from build123d import *
from build123d.topology import SkipClean

# Parameters (mm, degrees)
BASE_PLATE_DEPTH      = 15
SIDE_BLOCK_A_SKETCH_W = 40
SIDE_BLOCK_A_SKETCH_H = 15
SIDE_BLOCK_A_DEPTH    = 13.5
SIDE_BLOCK_B_SKETCH_W = 40
SIDE_BLOCK_B_SKETCH_H = 15
SIDE_BLOCK_B_DEPTH    = 13.5
UPRIGHT_WEB_SKETCH_W  = 46
UPRIGHT_WEB_SKETCH_H  = 10
UPRIGHT_WEB_DEPTH     = 25
LUG_EAR_DEPTH         = 10
LUG_HOLE_SKETCH_R     = 10
LUG_HOLE_DEPTH        = 10
GUSSET_DEPTH          = 46


with BuildPart() as part:
    # Base Plate Sketch → Base Plate (new body)
    with BuildSketch(Plane(origin=(0, 0, 0), x_dir=(1, 0, 0), z_dir=(0, 1, 0))):
        Polygon((13.5, 0), (13.5, 9.84759163), (32.5, 9.84759163), (32.5, 0), (46, 0), (46, 100), (0, 100), (0, 0), align=None)
    extrude(amount=BASE_PLATE_DEPTH)

    # Side Block A Sketch → Side Block A (add)
    with BuildSketch(Plane(origin=(0, 0, 0), x_dir=(0, 0, -1), z_dir=(1, 0, 0))):
        with Locations((50, -7.5)):
            Rectangle(SIDE_BLOCK_A_SKETCH_W, SIDE_BLOCK_A_SKETCH_H)
    extrude(amount=SIDE_BLOCK_A_DEPTH)

    # Side Block B Sketch → Side Block B (add)
    with BuildSketch(Plane(origin=(46, 0, 0), x_dir=(0, 0, -1), z_dir=(1, 0, 0))):
        with Locations((50, -7.5)):
            Rectangle(SIDE_BLOCK_B_SKETCH_W, SIDE_BLOCK_B_SKETCH_H)
    extrude(amount=-SIDE_BLOCK_B_DEPTH)

    # Upright Web Sketch → Upright Web (add)
    with BuildSketch(Plane(origin=(0, 15, 0), x_dir=(1, 0, 0), z_dir=(0, 1, 0))):
        with Locations((23, 55)):
            Rectangle(UPRIGHT_WEB_SKETCH_W, UPRIGHT_WEB_SKETCH_H)
    extrude(amount=UPRIGHT_WEB_DEPTH)

    # Lug Ear Sketch → Lug Ear (add)
    with BuildSketch(Plane.XY.offset(-50)):
        with BuildLine():
            ThreePointArc((33, 40), (23, 30), (13, 40))
            Line((13, 40), (0, 40))
            ThreePointArc((0, 40), (23, 17), (46, 40))
            Line((46, 40), (33, 40))
        make_face()
        with BuildLine():
            Line((0, 40), (13, 40))
            ThreePointArc((13, 40), (23, 50), (33, 40))
            Line((33, 40), (46, 40))
            ThreePointArc((46, 40), (23, 63), (0, 40))
        make_face()
    extrude(amount=-LUG_EAR_DEPTH)

    # Lug Hole Sketch → Lug Hole (cut)
    with SkipClean():  # the faces are left unmerged after this step: merging them gives an invalid solid
        with BuildSketch(Plane.XY.offset(-50)):
            with Locations((23, 40)):
                Circle(LUG_HOLE_SKETCH_R)
        extrude(amount=-LUG_HOLE_DEPTH, mode=Mode.SUBTRACT)

    # Gusset Sketch → Gusset (add)
    with SkipClean():  # the faces are left unmerged after this step: merging them gives an invalid solid
        with BuildSketch(Plane(origin=(46, 0, 0), x_dir=(0, 0, -1), z_dir=(1, 0, 0))):
            Polygon((50, 15), (24, 15), (50, 28), align=None)
        extrude(amount=-GUSSET_DEPTH)


solid = part.part
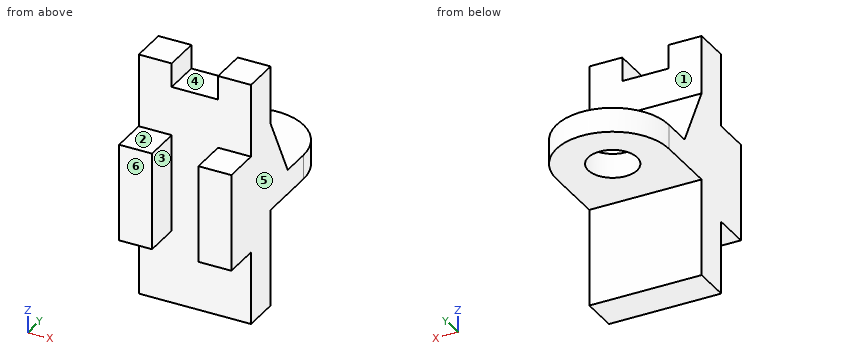
CAD build for the part. Positions are in the model's coordinates, mm. Face numbers are marked on the shaded views. A direction names the side the tool comes from. Coordinates: 2 decimals unless noted, no trailing zeros. Write each loop counter-clockwise with the first axis right and the second up, starting at its lowest first coordinate (ties: lowest second). Pieces come first, ordered by that corner, then holes. Notation, with made-up numbers: (44.5, 18) - (56.5, 18) arc R15 ccw to (56.5, 38) - close; hole circle Ø5 at (-35, 58.5). An arc over 180 degrees is marked (long way). Use a Markdown table: item, result. Add a question column.
Item 1: 3-axis set-ups, long thin cutter, end or side, ignore diameter. For the marked faces 1, 2 and 3: which of +Z, -Z, +X, -X, +Y, -Y reach the whole face in a straight line?
Item 2: Band-saw the part on C-C, the plane z = -47. Give the cut face in (x, y).
Item 3: Band-saw the part on D-D, the plane y = 35. Give the cut face in (x, z), and give its area (3 significant figures).
Item 4: Mould opens along X. For the marked faces 4, 5 and 6 say: pulls with the +X half, pulls with the -X half, needs draft (parallel to the pull), parting line crosses it, or undercut.
Item 5: Drill centre lines: L1, parallel to Y at x = 23, z = -58; L2, parallel to X at y = 11.5, z = -7; L3, parallel to Y at x = 26, z = -15.5. Where is each one in solid material? Low to high. Write a range as from..to.
Item 6: Flat gauge pins, fed straight in: pin 1 (7 mm diameter, centred on x = 8.5, y = -6.5, fed in from +Z); pin 2 (7.5 mm diameter, centred on x = 26.5, y = 9.5, fed in from +Z); pin 3 (12 mm diameter, centred on x = 18, z = -22, fed in from -Y); pin 4 (12 mm diameter, centred on x = 23, y = 40, fed in from +Z). Where does each tip first touch, or does it go through?
Item 7: Band-saw the part on A-A, the plane x = 23. Give the cut face in (y, z).
Item 8: Band-saw the part on B-B, the plane y = 3. Give the cut face in (x, z), and give its area (3 significant figures).
Numbers:
| question | item | result |
|---|---|---|
| 1 | face 1 | +Z, +X, -X, +Y |
| 1 | face 2 | +Z, +X, -X, -Y |
| 1 | face 3 | +Z, -Z, -Y |
| 2 | outline | (0, -15) - (13.5, -15) - (13.5, 0) - (32.5, 0) - (32.5, -15) - (46, -15) - (46, 26.5) - (0, 26.5) - close |
| 3 | outline | (0, -60) - (14.34, -60) - (14.34, -50) - (0, -50) - close; (31.66, -60) - (46, -60) - (46, -50) - (31.66, -50) - close |
| 3 | area | 287 mm2 |
| 4 | face 4 | undercut |
| 4 | face 5 | pulls with the +X half |
| 4 | face 6 | needs draft |
| 5 | L1 | 0..30, 50..63 |
| 5 | L2 | 0..13.5, 32.5..46 |
| 5 | L3 | 0..15 |
| 6 | pin 1 | z = -30 |
| 6 | pin 2 | z = -9.85 |
| 6 | pin 3 | y = 0 |
| 6 | pin 4 | through |
| 7 | outline | (0, -100) - (15, -100) - (15, -60) - (30, -60) - (30, -50) - (28, -50) - (15, -24) - (15, -9.85) - (0, -9.85) - close; (50, -60) - (63, -60) - (63, -50) - (50, -50) - close |
| 8 | outline | (0, -100) - (46, -100) - (46, 0) - (32.5, 0) - (32.5, -9.85) - (13.5, -9.85) - (13.5, 0) - (0, 0) - close |
| 8 | area | 4,410 mm2 |
